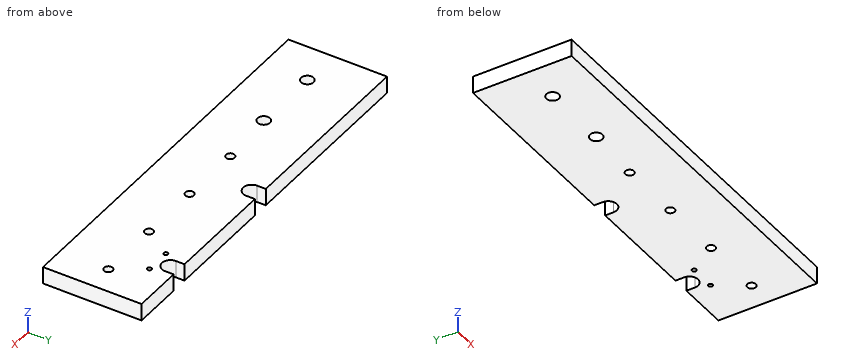
```python
from build123d import *

# Parameters (mm, degrees)
SKETCH1_W           = 900
SKETCH1_H           = 230
BOSS_EXTRUDE1_DEPTH = 20
SKETCH2_R           = 10
CUT_EXTRUDE1_DEPTH  = 467.181295206
CUT_EXTRUDE2_DEPTH  = 467.181295206
LPATTERN1_COUNT     = 2
LPATTERN1_PITCH     = 298
LPATTERN2_COUNT     = 4
LPATTERN2_PITCH     = 149
SKETCH5_R           = 5
CUT_EXTRUDE4_DEPTH  = 467.181295206
SKETCH6_R           = 14.5
CUT_EXTRUDE5_DEPTH  = 467.181295206


with BuildPart() as part:
    # Sketch1 → Boss-Extrude1 (new, symmetric)
    with BuildSketch(Plane.XY):
        Rectangle(SKETCH1_W, SKETCH1_H)
    extrude(amount=BOSS_EXTRUDE1_DEPTH, both=True)

    # Sketch2 → Cut-Extrude1 (cut, through all)
    with BuildSketch(Plane.XY.offset(20)):
        with Locations((387, -2.5)):
            Circle(SKETCH2_R)
    cut_extrude1 = extrude(amount=-CUT_EXTRUDE1_DEPTH, mode=Mode.SUBTRACT)

    # Sketch3 → Cut-Extrude2 (cut, through all)
    with BuildSketch(Plane.XY.offset(20)):
        with BuildLine():
            Line((332.5, 115), (332.5, 95))
            ThreePointArc((332.5, 95), (312.5, 75), (292.5, 95))
            Line((292.5, 95), (292.5, 115))
            ThreePointArc((292.5, 115), (312.5, 135), (332.5, 115))
        make_face()
    cut_extrude2 = extrude(amount=-CUT_EXTRUDE2_DEPTH, mode=Mode.SUBTRACT)

    # LPattern1: Cut-Extrude2 ×2
    with Locations(*[(-i * LPATTERN1_PITCH, 0, 0) for i in range(1, LPATTERN1_COUNT)]):
        add(cut_extrude2, mode=Mode.SUBTRACT)

    # LPattern2: Cut-Extrude1 ×4
    with Locations(*[(-i * LPATTERN2_PITCH, 0, 0) for i in range(1, LPATTERN2_COUNT)]):
        add(cut_extrude1, mode=Mode.SUBTRACT)

    # Sketch5 → Cut-Extrude4 (cut, through all)
    with BuildSketch(Plane(origin=(0, 0, -20), x_dir=(-1, 0, 0), z_dir=(0, 0, -1))):
        with Locations((-342.5, 65)):
            Circle(SKETCH5_R)
        with Locations(Location((-282.5, 65, 0), (0, 0, 180))):
            Circle(SKETCH5_R)
    extrude(amount=-CUT_EXTRUDE4_DEPTH, mode=Mode.SUBTRACT)

    # Sketch6 → Cut-Extrude5 (cut, through all)
    with BuildSketch(Plane(origin=(0, 0, -20), x_dir=(-1, 0, 0), z_dir=(0, 0, -1))):
        with Locations((356.1, -11)):
            Circle(SKETCH6_R)
        with Locations((196.1, -11)):
            Circle(SKETCH6_R)
    extrude(amount=-CUT_EXTRUDE5_DEPTH, mode=Mode.SUBTRACT)


solid = part.part
```
Here's how the part is built. I have some questions about the finished solid (model axes, mm). Coordinates: 2 decimals unless noted, no trailing zeros. Loops run counter-clockwise (first coordinate to the right, second up) from the corner with the lowest first, then second, coordinate; pieces in that order, holes last. Notation, with made-up numbers: (-5, -9.5) -> (3, -9.5) arc R9 ccw to (3, -1.5) -> close; hole circle Ø1 at (52, 49.25). An arc over 180 degrees is marked (long way). Return JSON: item names as keys, results as strings.
1) If we section it at A-A, the plane x = -196.1: Write out the boundary of the cut face in (y, z), then the cut area to 3 significant figures.
Results below:
{"outline": "(-115, -20) -> (-25.5, -20) -> (-25.5, 20) -> (-115, 20) -> close; (3.5, -20) -> (115, -20) -> (115, 20) -> (3.5, 20) -> close", "area": "8,040 mm²"}
2) If we section it at D-D, the plane x = 387: Write out the boundary of the cut face in (y, z), then the cut area to 3 significant figures.
Results below:
{"outline": "(-115, -20) -> (-12.5, -20) -> (-12.5, 20) -> (-115, 20) -> close; (7.5, -20) -> (115, -20) -> (115, 20) -> (7.5, 20) -> close", "area": "8,400 mm²"}
3) If we section it at B-B, the plane z = -13: Count the separate pieces of the cut face and the enclosed holes in it, then the cut area to 3 significant figures.
Results below:
{"separate pieces": "1", "enclosed holes": "8", "area": "201,000 mm²"}
4) Will this pin go through, and if not, where does the flat tip stop? pin 1 (18 mm diameter, centred on x = 387, y = -2.5, fed in from +Z).
Results below:
{"pin 1": "through"}
5) I need wall thicknesses on line 1 (X direction, y = 82, z = 9); line 2 (Y direction, x = 342.5, z = -0.5); line 3 (Y direction, x = -60, z = 10). Which ranges of each line are inside material? Lowest first, please. Write a range as from..to.
Results below:
{"line 1": "-450..-0.7, 29.7..297.3, 327.7..450", "line 2": "-115..60, 70..115", "line 3": "-115..-12.5, 7.5..115"}
6) If we section it at C-C, the plane y = 83.5: Write out the boundary of the cut face in (x, z).
Results below:
{"outline": "(-450, -20) -> (-1.86, -20) -> (-1.86, 20) -> (-450, 20) -> close; (30.86, -20) -> (296.14, -20) -> (296.14, 20) -> (30.86, 20) -> close; (328.86, -20) -> (450, -20) -> (450, 20) -> (328.86, 20) -> close"}
